Model file for the job. Use its own axes, mm. A direction names the side the tool comes from. Give positions to 0.01 mm unless a question says otherwise; leave off trailing zeros. Order: outer loops, then holes, each group sorted by start corner. A loop starts at its lowest first (then second) coordinate and runs counter-clockwise, first axis right, second up. Notation, with made-up numbers: M 58.25,-24 L 86.25,-24 A15 cw 86.25,-19 Z; hole C 57,87.5 d5. An arc over 180 degrees is marked long. Return JSON: item names as keys, results as strings. Group by question number.
1. Slice it at C-C on x = 158.5. List the corners of the cut face in (y, z), then the cut area to 3 significant figures.
2. 3-axis set-ups, long thin cutter, end or side, ignore diameter. For faces 1 (the face through (100, 15, -27)), 2 (the face through (114, 15, 0)), 3 (the face through (27, 15, 82)): which of +Z, -Z, +X, -X, +Y, -Y reach the whole face in a straight line?
3. Slice it at D-D on z = -10.5. List the corners of the cut face in (x, y), then the cut area to 3 significant figures.
4. Two-plate mould, pull along Y, no slides. Class faces 4 (the face through (28, 15, 170)), 5 (the face through (55, 30, -5)), 6 (the face through (3, 15, 70)): released by +Y, released by -Y, zero draft, split by the parting line, or undercut.
5. Wall check: probe 1 along Z at (x, y) = (192.5, 20); probe 2 along X at (y, z) = (26.75, 131). Give the ranges that are in metal, low to high. Write a range as [from, to].
6. Slice it at B-B on y = 24.5. List the corners of the cut face in (x, z).
7. Pin check, flat tips, straight feed: pin 1 (10 mm diameter, centred on y = 14.5, z = 37.5, fed in from +X); pin 2 (7 mm diameter, centred on x = 119, y = 16, fed in from +Z). Stop position of each tip, or through.
8. Slice it at A-A on z = 61. List the corners of the cut face in (x, y).
from build123d import *

# Parameters (mm, degrees)
SKETCH_1_W      = 200
SKETCH_1_H      = 30
EXTRUDE_1_DEPTH = 30
SKETCH_2_W      = 30
SKETCH_2_H      = 30
EXTRUDE_2_DEPTH = 170
SHELL_1_T       = -3


with BuildPart() as part:
    # 草图1 → 凸台-拉伸1 (new body)
    with BuildSketch(Plane.XY):
        with Locations((100, 15)):
            Rectangle(SKETCH_1_W, SKETCH_1_H)
    extrude(amount=-EXTRUDE_1_DEPTH)

    # 草图2 → 凸台-拉伸2 (add)
    with BuildSketch(Plane.XY):
        with Locations((15, 15)):
            Rectangle(SKETCH_2_W, SKETCH_2_H)
    extrude(amount=EXTRUDE_2_DEPTH)

    # 抽壳1
    shell_1_openings = [part.faces().sort_by_distance(p)[0] for p in [
        (15, 15, 170),
        (200, 15, -15),
    ]]
    offset(amount=SHELL_1_T, openings=shell_1_openings, kind=Kind.INTERSECTION)


solid = part.part
Result:
{
 "1": {"outline": "M 0,-30 L 30,-30 L 30,0 L 0,0 Z; hole M 3,-27 L 27,-27 L 27,-3 L 3,-3 Z", "area": "324 mm2"},
 "2": {"face 1": "+X", "face 2": "+Z, +X, +Y, -Y", "face 3": "+Z"},
 "3": {"outline": "M 0,0 L 200,0 L 200,3 L 3,3 L 3,27 L 200,27 L 200,30 L 0,30 Z", "area": "1,270 mm2"},
 "4": {"face 4": "zero draft", "face 5": "released by +Y", "face 6": "undercut"},
 "5": {"probe 1": "z = [-30, -27], [-3, 0]", "probe 2": "x = [0, 3], [27, 30]"},
 "6": {"outline": "M 0,-30 L 200,-30 L 200,-27 L 3,-27 L 3,170 L 0,170 Z; M 27,-3 L 200,-3 L 200,0 L 30,0 L 30,170 L 27,170 Z"},
 "7": {"pin 1": "stops at x = 30", "pin 2": "stops at z = 0"},
 "8": {"outline": "M 0,0 L 30,0 L 30,30 L 0,30 Z; hole M 3,3 L 27,3 L 27,27 L 3,27 Z"}
}
